Design review of the part built by this model. Coordinates are the model's own, in mm. Coordinates: 2 decimals unless noted, no trailing zeros. Loops run counter-clockwise (first coordinate to the right, second up) from the corner with the lowest first, then second, coordinate; pieces in that order, holes last. Notation, with made-up numbers: M 39,62.25 L 70,62.25 A12 ccw 70,76.25 Z; hole C 27.5,8 d5. An arc over 180 degrees is marked long. One line per item, written item: value.
```python
from build123d import *

# Parameters (mm, degrees)
SKETCH1_W           = 4.5
SKETCH1_H           = 3
BOSS_EXTRUDE1_DEPTH = 8
SKETCH2_W           = 2.9
SKETCH2_H           = 0.45
BOSS_EXTRUDE2_DEPTH = 26.5
FILLET1_R           = 0.5
CHAMFER1_SIZE       = 1
CHAMFER2_SIZE       = 0.1
SKETCH3_R           = 1.525
CUT_EXTRUDE1_DEPTH  = 2.1
SKETCH5_R           = 0.6
CUT_EXTRUDE2_DEPTH  = 2.1
CUT_EXTRUDE3_DEPTH  = 30.466082196
BOSS_EXTRUDE3_DEPTH = 3
SKETCH8_R           = 0.25
CUT_EXTRUDE4_DEPTH  = 3


with BuildPart() as part:
    # Sketch1 → Boss-Extrude1 (new body)
    with BuildSketch(Plane(origin=(0, 0, 0), x_dir=(1, 0, 0), z_dir=(0, 1, 0))):
        Rectangle(SKETCH1_W, SKETCH1_H)
    extrude(amount=BOSS_EXTRUDE1_DEPTH)

    # Sketch2 → Boss-Extrude2 (add)
    with BuildSketch(Plane.XY.offset(1.5)):
        with Locations((0, 0.425)):
            Rectangle(SKETCH2_W, SKETCH2_H)
    extrude(amount=BOSS_EXTRUDE2_DEPTH)

    # Fillet1
    fillet1_edges = [part.edges().sort_by_distance(p)[0] for p in [
        (1.45, 0.425, 28),
        (-1.45, 0.425, 28),
    ]]
    fillet(fillet1_edges, radius=FILLET1_R)

    # Chamfer1
    chamfer1_edges = [part.edges().sort_by_distance(p)[0] for p in [
        (0, 8, 1.5),
    ]]
    chamfer(chamfer1_edges, length=CHAMFER1_SIZE)

    # Chamfer2
    chamfer2_edges = [part.edges().sort_by_distance(p)[0] for p in [
        (0, 0.65, 28),
        (0, 0.2, 28),
        (1.45, 0.2, 14.5),
        (-1.45, 0.2, 14.5),
        (1.303553391, 0.2, 27.853553391),
        (-1.303553391, 0.2, 27.853553391),
        (-1.45, 0.65, 14.5),
        (1.45, 0.65, 14.5),
        (1.303553391, 0.65, 27.853553391),
        (-1.303553391, 0.65, 27.853553391),
    ]]
    chamfer(chamfer2_edges, length=CHAMFER2_SIZE)

    # Sketch3 → Cut-Extrude1 (cut)
    with BuildSketch(Plane.XY.offset(1.5)):
        with Locations((0, 3.825)):
            Circle(SKETCH3_R)
    extrude(amount=-CUT_EXTRUDE1_DEPTH, mode=Mode.SUBTRACT)

    # Sketch5 → Cut-Extrude2 (cut)
    with BuildSketch(Plane.XY.offset(-0.6)):
        with Locations((0, 3.825)):
            Circle(SKETCH5_R)
    extrude(amount=-CUT_EXTRUDE2_DEPTH, mode=Mode.SUBTRACT)

    # Sketch6 → Cut-Extrude3 (cut, through all)
    with BuildSketch(Plane(origin=(2.25, 0, 0), x_dir=(0, 0, -1), z_dir=(1, 0, 0))):
        Polygon((1.5, 8), (-0.5, 8), (-1.5, 7), (-1.5, 0), (1.5, 0), align=None)
    extrude(amount=-CUT_EXTRUDE3_DEPTH, mode=Mode.SUBTRACT)

    # Sketch7 → Boss-Extrude3 (add)
    with BuildSketch(Plane(origin=(0, 0, 1.5), x_dir=(-1, 0, 0), z_dir=(0, 0, -1))):
        Polygon((1.45, 0.55), (1.35, 0.65), (-1.35, 0.65), (-1.45, 0.55), (-1.45, 0.3), (-1.35, 0.2), (1.35, 0.2), (1.45, 0.3), align=None)
    extrude(amount=BOSS_EXTRUDE3_DEPTH)

    # Sketch8 → Cut-Extrude4 (cut)
    with BuildSketch(Plane.XZ.offset(-0.2)):
        with Locations(Location((0, -0.75, 0), (0, 0, 270))):
            Circle(SKETCH8_R)
    extrude(amount=-CUT_EXTRUDE4_DEPTH, mode=Mode.SUBTRACT)


solid = part.part
```
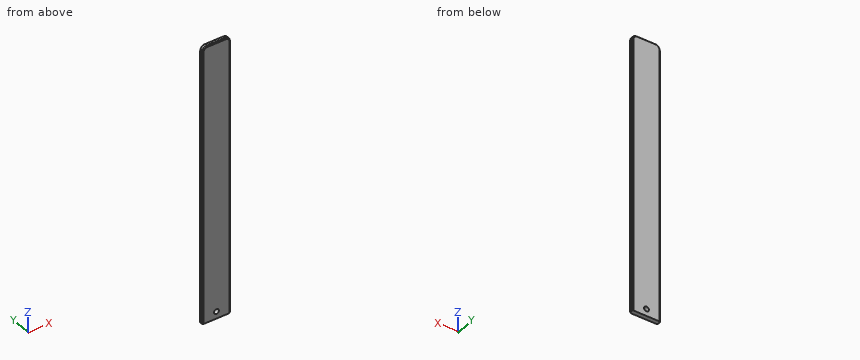
(1) We need section C-C on z = 20.25. State the section outline as (x, y) points.
Reply:
outline: M -1.45,0.3 L -1.35,0.2 L 1.35,0.2 L 1.45,0.3 L 1.45,0.55 L 1.35,0.65 L -1.35,0.65 L -1.45,0.55 Z
(2) We need section B-B on z = -0.75. State the section outline as (x, y) points, then the cut area to 3 significant figures.
Reply:
outline: M -1.45,0.3 L -1.35,0.2 L -0.25,0.2 L -0.25,0.65 L -1.35,0.65 L -1.45,0.55 Z; M 0.25,0.2 L 1.35,0.2 L 1.45,0.3 L 1.45,0.55 L 1.35,0.65 L 0.25,0.65 Z
area: 1.06 mm2
(3) We need section A-A on x = 0. State the section outline as (y, z) points.
Reply:
outline: M 0.2,-1.5 L 0.65,-1.5 L 0.65,-1 L 0.2,-1 Z; M 0.2,-0.5 L 0.65,-0.5 L 0.65,27.9 L 0.55,28 L 0.3,28 L 0.2,27.9 Z
(4) To check wall thickness, follow line 1 along X through (y, z) = (0.4, -0.75); line 2 along Z through (x, y) = (-1.25, 0.5); line 3 along Z through (x, y) = (0.05, 0.6). State the ranges of each line that lie inside material, in increasing order. Write a range as [from, to].
Reply:
line 1: x = [-1.45, -0.25], [0.25, 1.45]
line 2: z = [-1.5, 27.9]
line 3: z = [-1.5, -0.99], [-0.51, 27.95]
